```python
from build123d import *

# Parameters (mm, degrees)
BOSS_EXTRUDE1_DEPTH = 250
SKETCH2_W           = 86.5
SKETCH2_H           = 88.492592909
CUT_EXTRUDE1_DEPTH  = 250
SKETCH3_R           = 7.5
CUT_EXTRUDE2_DEPTH  = 250
CHAMFER1_SIZE       = 10


with BuildPart() as part:
    # Sketch1 → Boss-Extrude1 (new body)
    with BuildSketch(Plane.XY):
        with BuildLine():
            Line((0, 0), (-42, 0))
            ThreePointArc((-42, 0), (-51.192388155, -3.807611845), (-55, -13))
            Line((-55, -13), (-55, -200))
            Line((-55, -200), (-47, -200))
            Line((-47, -200), (-47, -13))
            ThreePointArc((-47, -13), (-45.535533906, -9.464466094), (-42, -8))
            Line((-42, -8), (0, -8))
            Line((0, -8), (0, 0))
        make_face()
    extrude(amount=BOSS_EXTRUDE1_DEPTH)

    # Sketch2 → Cut-Extrude1 (cut)
    with BuildSketch(Plane.ZY.offset(55)):
        Polygon((0, -50), (80, -200), (0, -200), align=None)
        Polygon((170, -200), (250, -200), (250, -50), align=None)
        with Locations((125, 28.246296455)):
            Rectangle(SKETCH2_W, SKETCH2_H)
    extrude(amount=-CUT_EXTRUDE1_DEPTH, mode=Mode.SUBTRACT)

    # Sketch3 → Cut-Extrude2 (cut)
    with BuildSketch(Plane(origin=(0, 0, 0), x_dir=(1, 0, 0), z_dir=(0, 1, 0))):
        with Locations(Location((-20, -20, 0), (0, 0, 180))):
            Circle(SKETCH3_R)
        with Locations(Location((-20, -230, 0), (0, 0, 180))):
            Circle(SKETCH3_R)
    extrude(amount=-CUT_EXTRUDE2_DEPTH, mode=Mode.SUBTRACT)

    # Chamfer1
    chamfer1_edges = [part.edges().sort_by_distance(p)[0] for p in [
        (0, -4, 250),
        (0, -4, 0),
    ]]
    chamfer(chamfer1_edges, length=CHAMFER1_SIZE)


solid = part.part
```
Build history of the part. All positions in model axes, mm. A direction names the side the tool comes from. Coordinates: 2 decimals unless noted, no trailing zeros. Write each loop counter-clockwise with the first axis right and the second up, starting at its lowest first coordinate (ties: lowest second). Pieces come first, ordered by that corner, then holes.
1. Band-saw the part on C-C, the plane y = -140. Give the cut face in (x, z).
Answer block:
outline: (-55, 48) - (-47, 48) - (-47, 202) - (-55, 202) - close
2. Drill centre lines: probe 1 along Z at (x, y) = (-20, -3.5); probe 2 along X at (y, z) = (-94, 85); probe 3 along Y at (x, z) = (-13, 38). Where is each one in solid material? Low to high.
Answer block:
probe 1: z = 0 to 12.5, 27.5 to 81.75, 168.25 to 222.5, 237.5 to 250
probe 2: x = -55 to -47
probe 3: y = -8 to 0
3. Band-saw the part on A-A, the plane x = -20. Give the cut face in (y, z), and give its area (3 significant figures).
Answer block:
outline: (-8, 0) - (0, 0) - (0, 12.5) - (-8, 12.5) - close; (-8, 27.5) - (0, 27.5) - (0, 81.75) - (-8, 81.75) - close; (-8, 168.25) - (0, 168.25) - (0, 222.5) - (-8, 222.5) - close; (-8, 237.5) - (0, 237.5) - (0, 250) - (-8, 250) - close
area: 1,070 mm2
4. Band-saw the part on D-D, the plane z = 175.5. Give the cut face in (x, y), and give its area (3 significant figures).
Answer block:
outline: (-55, -189.69) - (-47, -189.69) - (-47, -13) arc R5 cw to (-42, -8) - (0, -8) - (0, 0) - (-42, 0) arc R13 ccw to (-55, -13) - close
area: 1,860 mm2
5. Band-saw the part on B-B, the plane z = 230. Give the cut face in (x, y).
Answer block:
outline: (-55, -87.5) - (-47, -87.5) - (-47, -13) arc R5 cw to (-42, -8) - (-27.5, -8) - (-27.5, 0) - (-42, 0) arc R13 ccw to (-55, -13) - close; (-12.5, -8) - (0, -8) - (0, 0) - (-12.5, 0) - close
6. Drop flat-ended pins along their axis: pin 1 (6.5 mm diameter, centred on x = -51, z = 136, fed in from +Y); pin 2 (24 mm diameter, centred on x = -20, z = 230, fed in from +Y); pin 3 (1.5 mm diameter, centred on x = -30.5, z = 169.5, fed in from -Y); pin 4 (12 mm diameter, centred on y = -40, z = 215.5, fed in from +X). Give the stop position or say it passes through.
Answer block:
pin 1: stops at y = -16
pin 2: stops at y = 0
pin 3: stops at y = -8
pin 4: stops at x = -47
7. 3-axis set-ups, long thin cutter, end or side, ignore diameter. For faces 5 (the cylindrical face through (-19.024, -3.944, 237.436)), 6 (the flat face through (-47, -87, 123)), 7 (the flat face through (-28, -5, 168.25)): which of +Z, -Z, +X, -X, +Y, -Y reach the whole face in a straight line?
Answer block:
face 5: +Y, -Y
face 6: +Z, -Z, +X, -Y
face 7: +X, -X, +Y
8. Pull direction Z, two halves, no side cores. Call faces 1 (the cylindrical face through (-46, -10, 40)), 2 (the flat face through (-51, -16, 124)), 3 (the cylindrical face through (-14.5, -3.9, 25.1)), 4 (the flat face through (-48, -19, 0)): released by +Z, released by -Z, zero draft, split by the parting line, or undercut.
Answer block:
face 1: zero draft
face 2: undercut
face 3: undercut
face 4: released by -Z
